Read the model definition and answer for the solid it produces. Units are mm, in the model's axes. Face numbers are marked on the shaded views. A direction names the side the tool comes from. Coordinates: 2 decimals unless noted, no trailing zeros. Order: outer loops, then holes, each group sorted by start corner. A loop starts at its lowest first (then second) coordinate and runs counter-clockwise, first axis right, second up. Notation, with made-up numbers: M -4.75,-25 L 5.25,-25 A13 cw 5.25,-18 Z; hole C -3.75,53.5 d5. An arc over 180 degrees is marked long. Write each question's results on one line, items separated by ' | '.
```python
from build123d import *

# Parameters (mm, degrees)
SKETCH1_W           = 40
SKETCH1_H           = 40
BOSS_EXTRUDE1_DEPTH = 20
SKETCH2_W           = 6.5
SKETCH2_H           = 20
BOSS_EXTRUDE2_DEPTH = 2
SKETCH3_R           = 2
CUT_EXTRUDE1_DEPTH  = 2
SKETCH4_R           = 2
BOSS_EXTRUDE3_DEPTH = 4
FILLET1_R           = 2


with BuildPart() as part:
    # Sketch1 → Boss-Extrude1 (new body)
    with BuildSketch(Plane(origin=(0, 0, 0), x_dir=(1, 0, 0), z_dir=(0, 1, 0))):
        Rectangle(SKETCH1_W, SKETCH1_H)
    extrude(amount=BOSS_EXTRUDE1_DEPTH)

    # Sketch2 → Boss-Extrude2 (add)
    with BuildSketch(Plane(origin=(0, 0, 8), x_dir=(-1, 0, 0), z_dir=(0, 0, -1))):
        with Locations((23.25, 10)):
            Rectangle(SKETCH2_W, SKETCH2_H)
        with Locations((-23.25, 10)):
            Rectangle(SKETCH2_W, SKETCH2_H)
    extrude(amount=-BOSS_EXTRUDE2_DEPTH)

    # Sketch3 → Cut-Extrude1 (cut)
    with BuildSketch(Plane(origin=(0, 0, 8), x_dir=(-1, 0, 0), z_dir=(0, 0, -1))):
        with Locations((25.149376169, 5.012476611)):
            Circle(SKETCH3_R)
        with Locations((24.65, 15)):
            Circle(SKETCH3_R)
    cut_extrude1 = extrude(amount=-CUT_EXTRUDE1_DEPTH, mode=Mode.SUBTRACT)

    # Mirror2: Cut-Extrude1 across plane
    add(cut_extrude1.mirror(Plane.ZY), mode=Mode.SUBTRACT)

    # Sketch4 → Boss-Extrude3 (add)
    with BuildSketch(Plane.XY.offset(20)):
        with Locations(Location((-10, 10, 0), (0, 0, 180))):
            Circle(SKETCH4_R)
    extrude(amount=BOSS_EXTRUDE3_DEPTH)

    # Fillet1
    fillet1_edges = [part.edges().sort_by_distance(p)[0] for p in [
        (20, 20, -6),
        (20, 20, 15),
        (20, 0, -6),
        (20, 0, 15),
        (-20, 0, 15),
        (-20, 0, -6),
        (-20, 20, 15),
        (-20, 20, -6),
    ]]
    fillet(fillet1_edges, radius=FILLET1_R)


solid = part.part
```
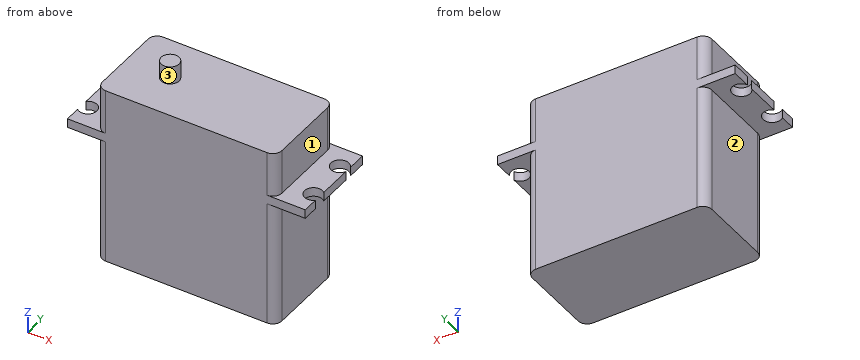
(1) The part is cut by section C-C, the plane z = 19. Write down the section's boundary in (x, y).
Conclusion:
outline: M -20,2 A2 ccw -18,0 L 18,0 A2 ccw 20,2 L 20,18 A2 ccw 18,20 L -18,20 A2 ccw -20,18 Z
(2) The part is cut by section D-D, the plane x = 5.5. Write down the section's boundary in (y, z).
Conclusion:
outline: M 0,-20 L 20,-20 L 20,20 L 0,20 Z
(3) Straight lines are drawn through the part: line 1 (Y direction, x = -24.65, z = 8.85); line 2 (Z direction, x = -18, y = 1.5). For each, find the intervals that lie inside material, in ascending order.
Conclusion:
line 1: 0 to 3.08, 6.95 to 13, 17 to 20 | line 2: -20 to 20
(4) The part is cut by section A-A, the plane x = 24.65. Write down the section's boundary in (y, z), then the cut area to 3 significant figures.
Conclusion:
outline: M 0,8 L 3.08,8 L 3.08,10 L 0,10 Z; M 6.95,8 L 13,8 L 13,10 L 6.95,10 Z; M 17,8 L 20,8 L 20,10 L 17,10 Z | area: 24.3 mm²
(5) The part is cut by section B-B, the plane y = 10. Write down the section's boundary in (x, z), then the cut area to 3 significant figures.
Conclusion:
outline: M -26.5,8 L -20,8 L -20,-20 L 20,-20 L 20,8 L 26.5,8 L 26.5,10 L 20,10 L 20,20 L -8,20 L -8,24 L -12,24 L -12,20 L -20,20 L -20,10 L -26.5,10 Z | area: 1,640 mm²
(6) For the marked faces 1, 2 and 3, determine the directions among +Z, -Z, +X, -X, +Y, -Y from which every point of the face is accessible in a straight line to the end or side of a thin tool.
Conclusion:
face 1: +Z, +X, +Y, -Y | face 2: -Z, -X, +Y, -Y | face 3: +Z
(7) Given pin 1 (2.5 mm diameter, centred on x = 23, y = 9.5, fed in from -Z); pin 2 (9.5 mm diameter, centred on x = -20.5, y = 14, fed in from +Z); pin 3 (3 mm diameter, centred on y = 11.5, z = 15, fed in from -X), each flat-ended and moving along its own axis, determine where each tip first touches the part or whether it passes through.
Conclusion:
pin 1: z = 8 | pin 2: z = 20 | pin 3: x = -20
